from build123d import *

# Parameters (mm, degrees)
SKETCH1_R               = 45
SKETCH1_R_2             = 30
BOSS_EXTRUDE1_DEPTH     = 34
CUT_EXTRUDE1_DEPTH      = 73.15261603
CUT_EXTRUDE1_DEPTH_BACK = 73.15261603
SKETCH3_R               = 6.5
CHAMFER1_SIZE           = 5
CHAMFER2_SIZE           = 3


with BuildPart() as part:
    # Sketch1 → Boss-Extrude1 (new body)
    with BuildSketch(Plane.XY):
        Circle(SKETCH1_R)
        Circle(SKETCH1_R_2, mode=Mode.SUBTRACT)
    extrude(amount=BOSS_EXTRUDE1_DEPTH)

    # Sketch3 → Cut-Extrude1 (cut, two sides: drawn at the far end of the back side and taken through both)
    with BuildSketch(Plane(origin=(0, 0, 0), x_dir=(1, 0, 0), z_dir=(0, 1, 0)).offset(-CUT_EXTRUDE1_DEPTH_BACK)):
        with Locations(Location((0, -17, 0), (0, 0, 270))):
            Circle(SKETCH3_R)
    extrude(amount=CUT_EXTRUDE1_DEPTH + CUT_EXTRUDE1_DEPTH_BACK, mode=Mode.SUBTRACT)

    # Chamfer1
    chamfer1_edges = [part.edges().sort_by_distance(p)[0] for p in [
        (-45, 0, 34),
    ]]
    chamfer(chamfer1_edges, length=CHAMFER1_SIZE)

    # Chamfer2
    chamfer2_edges = [part.edges().sort_by_distance(p)[0] for p in [
        (-45, 0, 0),
    ]]
    chamfer(chamfer2_edges, length=CHAMFER2_SIZE)


solid = part.part
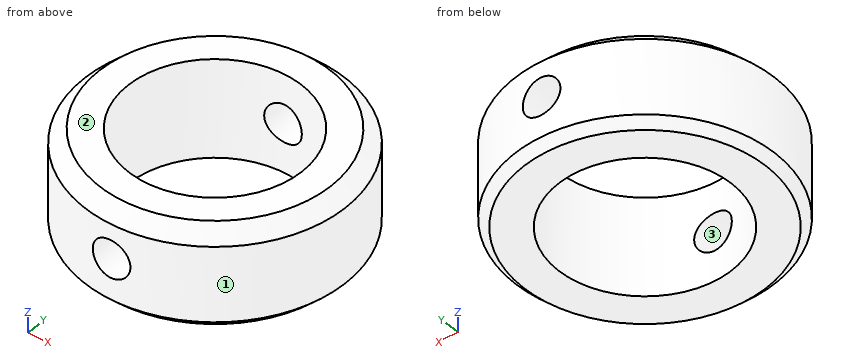
CAD build for the part. Positions are in the model's coordinates, mm. Face numbers are marked on the shaded views. Give positions to 0.01 mm unless a question says otherwise; leave off trailing zeros. Loops run counter-clockwise (first coordinate to the right, second up) from the corner with the lowest first, then second, coordinate; pieces in that order, holes last. Notation, with made-up numbers: M 76.25,61.5 L 100.25,61.5 A29 ccw 100.25,100.5 Z; hole C 50,-21.5 d3. An arc over 180 degrees is marked long. One line per question, with ' | ' between items. Start each with the question number.
1. Saw through at B-B on x = 0. Give the cut face in (y, z).
2. Saw through at C-C on z = 14. Give the cut face in (x, y).
3. Two-plate mould, pull along X, no slides. Class the marked faces 1, 2 and 3: pulls with the +X half, pulls with the -X half, needs draft (parallel to the pull), parting line crosses it, or undercut.
4. Flat gauge pins, fed straight in: pin 1 (3 mm diameter, centred on y = -21.5, z = 28, fed in from +X); pin 2 (5 mm diameter, centred on y = -28, z = 10.5, fed in from -X); pin 3 (1.5 mm diameter, centred on x = -30.5, z = 23.5, fed in from -Y). Where does each tip first touch, or does it go through?
5. Saw through at A-A on y = 0. Give the cut face in (x, z).
6. Probe L1, parallel to Y at x = 0, z = 7.5; L2, parallel to Z at x = 0, y = 35.5; L3, parallel to Y at x = -5, z = 10. List the from-to ranges inside material, lowest first. Write a range as from..to.
Result sheet:
1) outline: M -45,3 L -42,0 L -30,0 L -30,10.5 L -45,10.5 Z; M -45,23.5 L -30,23.5 L -30,34 L -40,34 L -45,29 Z; M 30,0 L 42,0 L 45,3 L 45,10.5 L 30,10.5 Z; M 30,23.5 L 45,23.5 L 45,29 L 40,34 L 30,34 Z
2) outline: M -5.77,-44.63 L -5.77,-29.44 A30 cw -5.77,29.44 L -5.77,44.63 A45 ccw Z; M 5.77,-44.63 A45 ccw 5.77,44.63 L 5.77,29.44 A30 cw 5.77,-29.44 Z
3) face 1: parting line crosses it | face 2: needs draft | face 3: undercut
4) pin 1: stops at x = 40.31 | pin 2: stops at x = -37.08 | pin 3: stops at y = -33.76
5) outline: M -45,3 L -42,0 L -30,0 L -30,34 L -40,34 L -45,29 Z; M 30,0 L 42,0 L 45,3 L 45,29 L 40,34 L 30,34 Z
6) L1: y = -45..-30, 30..45 | L2: z = 0..10.5, 23.5..34 | L3: y = -44.72..-29.58, 29.58..44.72
